Source: three-view drawing plus pictorial views. Frame: mm from the lowest corner of the part. A direction names the side the tool comes from. Round coordinates to 2 decimals unless told otherwise and drop trailing zeros. Loops run counter-clockwise (first coordinate to the right, second up) from the corner with the lowest first, then second, coordinate; pieces in that order, holes last. Notation, with made-up numbers: (-39, -3) -> (-8, -3) arc R3 cw to (-8, 1) -> close; hole circle Ø6 at (-4, -27.75). An arc over 180 degrees is marked (long way). One line per question, with ' | ' between items. Start each with the question number.
Q1. Contact query for flat-ended pins moving along their axis: P1, Ø12, axis at x = 71.5, z = 64.5, coming from the +Y side; P2, Ø18.5, axis at y = 80, z = 15, coming from the +X side; P3, Ø8, axis at y = 58, z = 58, coming from the -X side; P4, Ø2, axis at x = 22, y = 67, coming from the -Z side. Output: stop coordinate, or through.
Q2. Mould query, pull axis X, two halves, no side actions, for the marked faces 4, 5 and 6. Classes: pulls with the +X half, pulls with the -X half, needs draft (parallel to the pull), parting line crosses it, or undercut.
Q3. Cut plane D-D on x = 40. Return loops of the section in (y, z), and give its area (3 significant figures).
Q4. Cut plane B-B on z = 85. Return loops of the section in (x, y).
Q5. Cut plane C-C on y = 38.5. Return loops of the section in (x, z) (1 decimal).
Q6. Material intervals for L1, parallel to X at y = 54.5, z = 25; L2, parallel to Y at x = 58, z = 72; L3, parallel to Y at x = 54, z = 54 (1 decimal), sorted ascending.
Q7. Access query for the marked faces 1, 2 and 3. Directions: +Z, -Z, +X, -X, +Y, -Y. A direction counts if a zero-diameter tool reaches every point of the face in a straight line with its end or side. Return the directions, or none.
Q8. Cut plane A-A on x = 10. Return loops of the section in (y, z), and give its area (3 significant figures).
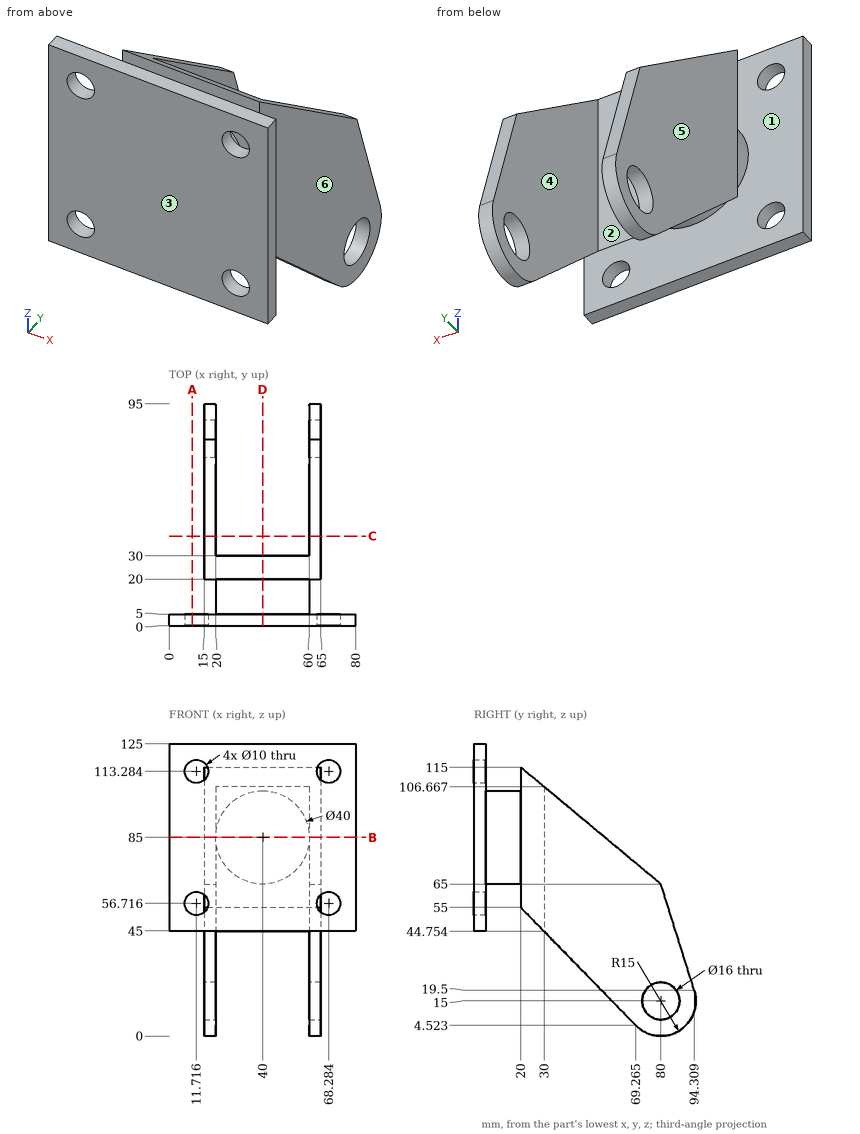
Results:
1) P1: y = 5 | P2: x = 65 | P3: x = 15 | P4: through
2) face 4: undercut | face 5: pulls with the -X half | face 6: pulls with the +X half
3) outline: (0, 45) -> (5, 45) -> (5, 65) -> (20, 65) -> (20, 55) -> (30, 44.75) -> (30, 106.67) -> (20, 115) -> (20, 105) -> (5, 105) -> (5, 125) -> (0, 125) -> close | area: 1,610 mm^2
4) outline: (0, 0) -> (80, 0) -> (80, 5) -> (60, 5) -> (60, 20) -> (65, 20) -> (65, 56) -> (60, 56) -> (60, 30) -> (20, 30) -> (20, 56) -> (15, 56) -> (15, 20) -> (20, 20) -> (20, 5) -> (0, 5) -> close
5) outline: (15, 36) -> (20, 36) -> (20, 99.6) -> (15, 99.6) -> close; (60, 36) -> (65, 36) -> (65, 99.6) -> (60, 99.6) -> close
6) L1: 15 to 20, 60 to 65 | L2: 0 to 5, 20 to 30 | L3: 0 to 5, 21 to 30
7) face 1: none | face 2: +Z, -Z, +Y | face 3: +Z, -Z, +X, -X, -Y
8) outline: (0, 45) -> (5, 45) -> (5, 52.02) -> (0, 52.02) -> close; (0, 61.41) -> (5, 61.41) -> (5, 108.59) -> (0, 108.59) -> close; (0, 117.98) -> (5, 117.98) -> (5, 125) -> (0, 125) -> close | area: 306 mm^2
